Could you check a few things on this model? Use its own coordinates, in mm. Face numbers are marked on the shaded views. Coordinates: 2 decimals unless noted, no trailing zeros. Loops run counter-clockwise (first coordinate to the right, second up) from the corner with the lowest first, then second, coordinate; pieces in that order, holes last.
1) Imagine slicing it at D-D on y = 9.5. Please give me the cut outline in (x, z), plus the area to 3 significant figures.
2) Thinking about a two-plate mould opening in X: for the marked faces 1, 2 and 3, which applies, released by +X, released by -X, zero draft, split by the parting line, or undercut?
3) If I drill on line 1 along Z through (x, y) = (0, 7.25); line 2 along Z through (x, y) = (3.25, 7.5), over which ranges is the centre line in solid material (lowest first)?
4) Imagine slicing it at A-A on z = 0. Please give me the cut outline in (x, y).
5) Imagine slicing it at C-C on y = 19.5. Please give me the cut outline in (x, z).
6) Will these pins go through, and if not, where does the flat tip stop? P1, Ø8, axis at y = 8, z = -8.5, coming from the +X side; P2, Ø6.5, axis at x = 0, z = 0, coming from the -Y side; P3, Ø1.5, axis at x = -1.5, y = 11.5, coming from the -Z side; P4, Ø1.5, axis at y = 19.5, z = -1, coming from the -X side.
7) Imagine slicing it at B-B on x = 0. Please give me the cut outline in (y, z), plus the area to 3 significant figures.
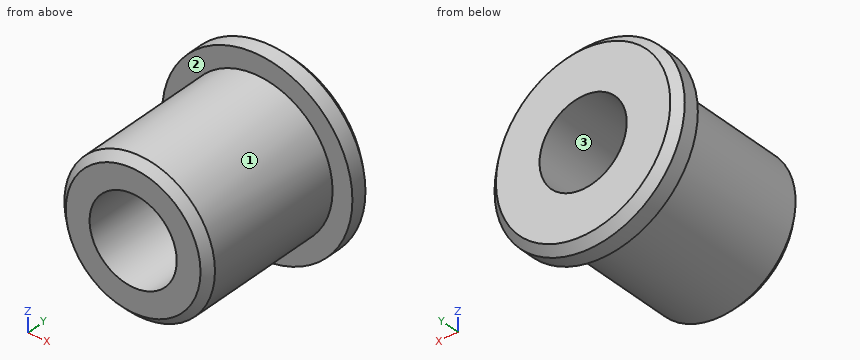
```python
from build123d import *

# Parameters (mm, degrees)
CUT_EXTRUDE_1_DEPTH      = 28.784887979
CUT_EXTRUDE_1_DEPTH_BACK = 28.784887979
SKETCH_2_R               = 5.5
CHAMFER_1_SIZE           = 1
CHAMFER_2_SIZE           = 1


with BuildPart() as part:
    # 草图1 → 旋转1 (revolve)
    with BuildSketch(Plane.XY):
        Polygon((0, 0), (0, 22), (12, 22), (12, 19), (9.5, 19), (9.5, 0), align=None)
    revolve(axis=Axis((0, 0, 0), (0, 1, 0)))

    # 草图2 → 切除-拉伸1 (cut, two sides: drawn at the far end of the back side and taken through both)
    with BuildSketch(Plane.XZ.offset(-CUT_EXTRUDE_1_DEPTH_BACK)):
        with Locations(Location((0, 0, 0), (0, 0, 270))):
            Circle(SKETCH_2_R)
    extrude(amount=CUT_EXTRUDE_1_DEPTH + CUT_EXTRUDE_1_DEPTH_BACK, mode=Mode.SUBTRACT)

    # 倒角1
    chamfer_1_edges = [part.edges().sort_by_distance(p)[0] for p in [
        (-12, 22, 0),
    ]]
    chamfer(chamfer_1_edges, length=CHAMFER_1_SIZE)

    # 倒角2
    chamfer_2_edges = [part.edges().sort_by_distance(p)[0] for p in [
        (-9.5, 0, 0),
    ]]
    chamfer(chamfer_2_edges, length=CHAMFER_2_SIZE)


solid = part.part
```
Filled in:
1. outline: circle Ø19 at (0, 0); hole circle Ø11 at (0, 0)
1. area: 188 mm2
2. face 1: split by the parting line
2. face 2: zero draft
2. face 3: undercut
3. line 1: z = -9.5 to -5.5, 5.5 to 9.5
3. line 2: z = -8.93 to -4.44, 4.44 to 8.93
4. outline: (-12, 19) - (-9.5, 19) - (-9.5, 1) - (-8.5, 0) - (-5.5, 0) - (-5.5, 22) - (-11, 22) - (-12, 21) - close; (5.5, 0) - (8.5, 0) - (9.5, 1) - (9.5, 19) - (12, 19) - (12, 21) - (11, 22) - (5.5, 22) - close
5. outline: circle Ø24 at (0, 0); hole circle Ø11 at (0, 0)
6. P1: stops at x = 8.37
6. P2: passes through
6. P3: stops at z = -9.47
6. P4: stops at x = -12
7. outline: (0, -8.5) - (1, -9.5) - (19, -9.5) - (19, -12) - (21, -12) - (22, -11) - (22, -5.5) - (0, -5.5) - close; (0, 5.5) - (22, 5.5) - (22, 11) - (21, 12) - (19, 12) - (19, 9.5) - (1, 9.5) - (0, 8.5) - close
7. area: 189 mm2
